```python
from build123d import *

# Parameters (mm, degrees)
SKETCH1_R           = 32
BOSS_EXTRUDE1_DEPTH = 3
SKETCH2_R           = 20
BOSS_EXTRUDE2_DEPTH = 3
SKETCH3_R           = 17
CUT_EXTRUDE1_DEPTH  = 1.5
SKETCH4_R           = 2.5
CUT_EXTRUDE2_DEPTH  = 36.5
CHAMFER1_SIZE       = 0.5


with BuildPart() as part:
    # Sketch1 → Boss-Extrude1 (new body)
    with BuildSketch(Plane(origin=(0, 0, 0), x_dir=(0, 0, -1), z_dir=(1, 0, 0))):
        Circle(SKETCH1_R)
    extrude(amount=BOSS_EXTRUDE1_DEPTH)

    # Sketch2 → Boss-Extrude2 (add)
    with BuildSketch(Plane(origin=(3, 0, 0), x_dir=(0, 0, -1), z_dir=(1, 0, 0))):
        Circle(SKETCH2_R)
    extrude(amount=BOSS_EXTRUDE2_DEPTH)

    # Sketch3 → Cut-Extrude1 (cut)
    with BuildSketch(Plane(origin=(6, 0, 0), x_dir=(0, 0, -1), z_dir=(1, 0, 0))):
        Circle(SKETCH3_R)
    extrude(amount=-CUT_EXTRUDE1_DEPTH, mode=Mode.SUBTRACT)

    # Sketch4 → Cut-Extrude2 (cut)
    with BuildSketch(Plane.ZY):
        with Locations((0, 25)):
            Circle(SKETCH4_R)
        with Locations((21.650635095, -12.5)):
            Circle(SKETCH4_R)
        with Locations((-21.650635095, -12.5)):
            Circle(SKETCH4_R)
    extrude(amount=-CUT_EXTRUDE2_DEPTH, mode=Mode.SUBTRACT)

    # Chamfer1
    chamfer1_edges = [part.edges().sort_by_distance(p)[0] for p in [
        (0, 0, 32),
        (6, 0, 20),
    ]]
    chamfer(chamfer1_edges, length=CHAMFER1_SIZE)


solid = part.part
```
Could you check a few things on this model? Use its own coordinates, in mm. A direction names the side the tool comes from. Give positions to 0.01 mm unless a question says otherwise; leave off trailing zeros. Order: outer loops, then holes, each group sorted by start corner. A loop starts at its lowest first (then second) coordinate and runs counter-clockwise, first axis right, second up.
Q1. We'd pull the mould along Y, two halves only. Please class faces 3 (the cylindrical face through (1.48, -13.46, 23.96)), 4 (the cylindrical face through (4.232, -19.524, 4.336)), 5 (the flat face through (6, 17.4, -1.4)): +Y half, -Y half, draft (parallel to the pull), parting line (faces both ways), or undercut.
Q2. Suppose I cut it at C-C, the plane x = 1.3. Write out the boundary of the cut face in (y, z).
Q3. For faces 1 (the cylindrical face through (5.26, 14.334, -9.139)), 2 (the cylindrical face through (1.48, -14.94, -22.19)), which set-ups out of +Z, -Z, +X, -X, +Y, -Y let a thin tool reach every point of the face, with its end or its side?
Q4. If I drill on line 1 along Y through (x, z) = (0.8, 0); line 2 along Y through (x, z) = (1.5, 0.5); line 3 along Z through (x, y) = (1.85, 24), over which ranges is the centre line in solid material (lowest first)?
Q5. Suppose I cut it at A-A, the plane z = 0. Write out the boundary of the cut face in (x, y).
Q6. Suppose I cut it at B-B, the plane y = 0. Write out the boundary of the cut face in (x, z).
Q7. Suppose I cut it at D-D, the plane y = -12.5. Count the separate pieces of the cut face and the enclosed holes in it, and give its area (3 significant figures).
Q8. I'm going to push flat-ended pins straight in: P1, Ø5, axis at y = 1.5, z = -20.5, coming from the +X side; P2, Ø1, axis at x = 1, y = -20, coming from the -Z side; P3, Ø3, axis at x = 1, y = -2, coming from the -Z side; P4, Ø6.5, axis at y = -12.5, z = 21.65, coming from the +X side. Where does each tip first touch, or does it pass through?
Solution:
1. face 3: undercut
1. face 4: parting line
1. face 5: draft
2. outline: circle Ø64 at (0, 0); hole circle Ø5 at (-12.5, -21.65); hole circle Ø5 at (-12.5, 21.65); hole circle Ø5 at (25, 0)
3. face 1: +X
3. face 2: +X, -X
4. line 1: y = -32 to 22.5, 27.5 to 32
4. line 2: y = -32 to 22.55, 27.45 to 32
4. line 3: z = -21.17 to -2.29, 2.29 to 21.17
5. outline: (0, -31.5) - (0.5, -32) - (3, -32) - (3, -20) - (5.5, -20) - (6, -19.5) - (6, -17) - (4.5, -17) - (4.5, 17) - (6, 17) - (6, 19.5) - (5.5, 20) - (3, 20) - (3, 22.5) - (0, 22.5) - close; (0, 27.5) - (3, 27.5) - (3, 32) - (0.5, 32) - (0, 31.5) - close
6. outline: (0, -31.5) - (0.5, -32) - (3, -32) - (3, -20) - (5.5, -20) - (6, -19.5) - (6, -17) - (4.5, -17) - (4.5, 17) - (6, 17) - (6, 19.5) - (5.5, 20) - (3, 20) - (3, 32) - (0.5, 32) - (0, 31.5) - close
7. separate pieces: 3
7. enclosed holes: 0
7. area: 205 mm2
8. P1: stops at x = 6
8. P2: stops at z = -25.37
8. P3: stops at z = -32
8. P4: stops at x = 3
